The figure shows three views and two pictorial views of one solid part (mm, origin at its lowest corner). Answer the questions. A direction names the side the tool comes from. Coordinates: 2 decimals unless noted, no trailing zeros. Write each loop counter-clockwise with the first axis right and the second up, starting at its lowest first coordinate (ties: lowest second). Pieces come first, ordered by that corner, then holes.
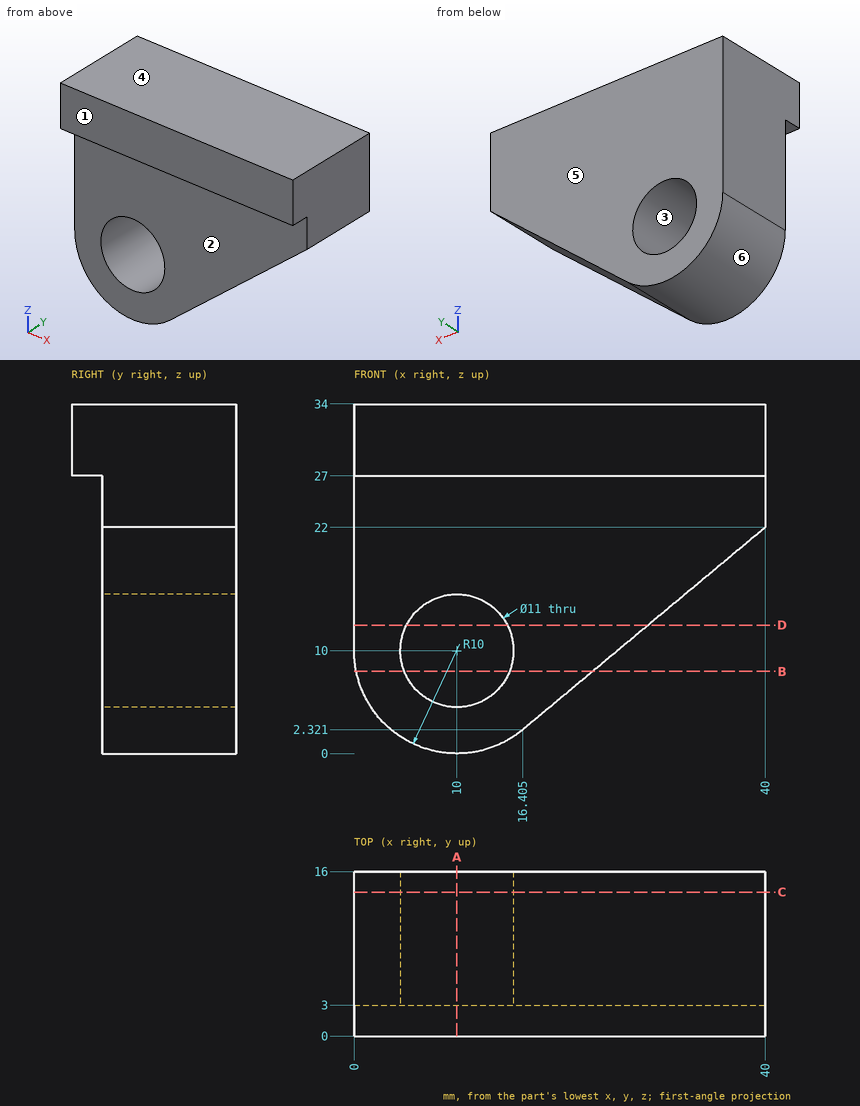
Q1. Which of the six approach directions +Z, -Z, +X, -X, +Y, -Y give full straight-line access (tool end or side, diameter ignored) to the marked faces 1 and 2?
Answers below:
face 1: +Z, -Z, +X, -X, -Y
face 2: -Z, +X, -X, -Y
Q2. Determine the mould class of the marked faces 3, 4, 5 and 6 for opening direction Z: released by +Z, released by -Z, zero draft, split by the parting line, or undercut.
Answers below:
face 3: undercut
face 4: released by +Z
face 5: zero draft
face 6: released by -Z
Q3. The part is cut by section C-C, the plane y = 14. Write down the section's boundary in (x, z) (1 decimal), then the cut area to 3 significant figures.
Answers below:
outline: (0, 10) arc R10 ccw to (16.4, 2.3) - (40, 22) - (40, 34) - (0, 34) - close; hole circle Ø11 at (10, 10)
area: 952 mm2
Q4. The part is cut by section D-D, the plane z = 12.5. Write down the section's boundary in (x, y).
Answers below:
outline: (0, 3) - (5.1, 3) - (5.1, 16) - (0, 16) - close; (14.9, 3) - (28.61, 3) - (28.61, 16) - (14.9, 16) - close
Q5. The part is cut by section B-B, the plane z = 8. Write down the section's boundary in (x, y) (1 decimal), then the cut area to 3 significant figures.
Answers below:
outline: (0.2, 3) - (4.9, 3) - (4.9, 16) - (0.2, 16) - close; (15.1, 3) - (23.2, 3) - (23.2, 16) - (15.1, 16) - close
area: 166 mm2
Q6. The part is cut by section A-A, the plane x = 10. Write down the section's boundary in (y, z), then the cut area to 3 significant figures.
Answers below:
outline: (0, 27) - (3, 27) - (3, 15.5) - (16, 15.5) - (16, 34) - (0, 34) - close; (3, 0) - (16, 0) - (16, 4.5) - (3, 4.5) - close
area: 320 mm2
Q7. Find the intervals of material crossed by probe 1 along X at (y, z) = (12.5, 8.5) (1 decimal); probe 2 along Y at (x, z) = (5.5, 15); probe 3 along X at (y, z) = (12.75, 6.5) (1 decimal), in increasing order.
Answers below:
probe 1: x = 0.1 to 4.7, 15.3 to 23.8
probe 2: y = 3 to 16
probe 3: x = 0.6 to 5.8, 14.2 to 21.4
Q8. Given pin 1 (8 mm diameter, centred on y = 7, z = 12.5, fed in from +X) (1 decimal); pin 2 (8 mm diameter, centred on x = 17, z = 13, fed in from -Y); pin 3 (0.9 mm diameter, centred on x = 27.5, y = 2, fed in from -Z), each flat-ended and moving along its own axis, determine where each tip first touches the part or whether it passes through.
Answers below:
pin 1: stops at x = 33.4
pin 2: stops at y = 3
pin 3: stops at z = 27
